Can you work these out from the model? Positions are in its coordinate system, mm. Give positions to 0.01 mm unless a question says otherwise; leave off trailing zeros. Order: outer loops, then holes, each group sorted by start corner. A loop starts at its lowest first (then second) coordinate and runs counter-clockwise, first axis right, second up. Notation, with made-up numbers: (-15, -26) -> (-7, -26) arc R15 ccw to (-7, -5) -> close; hole circle Ø2 at (45, 18). An arc over 180 degrees is marked (long way). Answer as CSV lines item,"result".
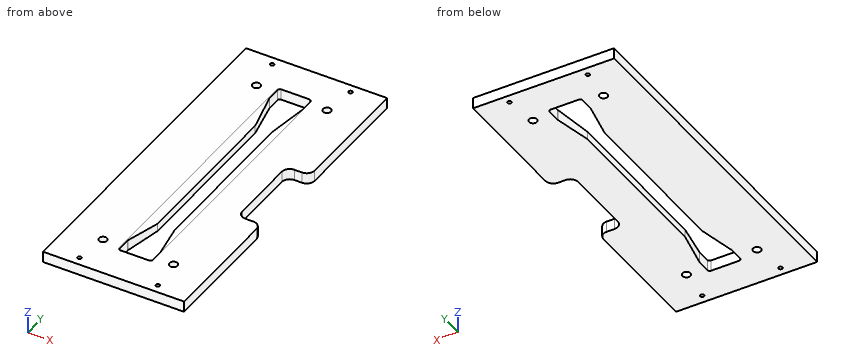
```python
from build123d import *

# Parameters (mm, degrees)
SKETCH1_W              = 180
SKETCH1_H              = 436
BOSS_EXTRUDE1_DEPTH    = 14
SKETCH5_W              = 30
SKETCH5_H              = 105
CUT_EXTRUDE1_DEPTH     = 472.902532309
M12_TAPPED_HOLE1_D     = 10.2
M12_TAPPED_HOLE1_DEPTH = 32.75
M12_TAPPED_HOLE1_TIP   = 3.064389157
FILLET1_R              = 10
M6_TAPPED_HOLE1_D      = 5
M6_TAPPED_HOLE1_DEPTH  = 17
M6_TAPPED_HOLE1_TIP    = 1.502151548
CUT_EXTRUDE2_DEPTH     = 5
CUT_EXTRUDE2_DRAFT     = -70


with BuildPart() as part:
    # Sketch1 → Boss-Extrude1 (new body)
    with BuildSketch(Plane.XY):
        with Locations((90, 218)):
            Rectangle(SKETCH1_W, SKETCH1_H)
        with BuildLine():
            Line((72, 45.5), (108, 45.5))
            ThreePointArc((108, 45.5), (110.121320344, 46.378679656), (111, 48.5))
            Line((111, 48.5), (111, 65.187634121))
            ThreePointArc((111, 65.187634121), (110.98386897, 65.498320406), (110.935649355, 65.805665564))
            Line((110.935649355, 65.805665564), (101, 113))
            Line((101, 113), (101, 323))
            Line((101, 323), (110.935649355, 370.194334436))
            ThreePointArc((110.935649355, 370.194334436), (110.98386897, 370.501679594), (111, 370.812365879))
            Line((111, 370.812365879), (111, 387.5))
            ThreePointArc((111, 387.5), (110.121320344, 389.621320344), (108, 390.5))
            Line((108, 390.5), (72, 390.5))
            ThreePointArc((72, 390.5), (69.878679656, 389.621320344), (69, 387.5))
            Line((69, 387.5), (69, 370.812365879))
            ThreePointArc((69, 370.812365879), (69.01613103, 370.501679594), (69.064350645, 370.194334436))
            Line((69.064350645, 370.194334436), (79, 323))
            Line((79, 323), (79, 113))
            Line((79, 113), (69.064350645, 65.805665564))
            ThreePointArc((69.064350645, 65.805665564), (69.01613103, 65.498320406), (69, 65.187634121))
            Line((69, 65.187634121), (69, 48.5))
            ThreePointArc((69, 48.5), (69.878679656, 46.378679656), (72, 45.5))
        make_face(mode=Mode.SUBTRACT)
    extrude(amount=-BOSS_EXTRUDE1_DEPTH)

    # Sketch5 → Cut-Extrude1 (cut, through all)
    with BuildSketch(Plane.XY):
        with Locations((165, 218)):
            Rectangle(SKETCH5_W, SKETCH5_H)
    extrude(amount=-CUT_EXTRUDE1_DEPTH, mode=Mode.SUBTRACT)

    # M12 Tapped Hole1
    with Locations(Plane(origin=(0, 0, -14), x_dir=(-1, 0, 0), z_dir=(0, 0, -1))):
        with Locations((-135, 383), (-45, 383), (-45, 53), (-135, 53)):
            Hole(M12_TAPPED_HOLE1_D / 2, depth=M12_TAPPED_HOLE1_DEPTH)
            with Locations((0, 0, -(M12_TAPPED_HOLE1_DEPTH + M12_TAPPED_HOLE1_TIP / 2))):  # 118° drill point
                Cone(0, M12_TAPPED_HOLE1_D / 2, M12_TAPPED_HOLE1_TIP, mode=Mode.SUBTRACT)

    # Fillet1
    fillet1_edges = [part.edges().sort_by_distance(p)[0] for p in [
        (150, 165.5, -7),
        (150, 270.5, -7),
        (180, 270.5, -7),
        (180, 165.5, -7),
    ]]
    fillet(fillet1_edges, radius=FILLET1_R)

    # M6 Tapped Hole1
    with Locations(Plane.XY):
        with Locations((40, 425), (140, 425), (40, 11), (140, 11)):
            Hole(M6_TAPPED_HOLE1_D / 2, depth=M6_TAPPED_HOLE1_DEPTH)
            with Locations((0, 0, -(M6_TAPPED_HOLE1_DEPTH + M6_TAPPED_HOLE1_TIP / 2))):  # 118° drill point
                Cone(0, M6_TAPPED_HOLE1_D / 2, M6_TAPPED_HOLE1_TIP, mode=Mode.SUBTRACT)


with BuildPart() as cut_extrude2_tool:
    # Sketch8 → Cut-Extrude2 (with draft: the straight prism first)
    with BuildSketch(Plane.XY):
        with BuildLine():
            ThreePointArc((71, 390.5), (68.878679656, 389.621320344), (68, 387.5))
            Line((68, 387.5), (68, 48.5))
            ThreePointArc((68, 48.5), (68.878679656, 46.378679656), (71, 45.5))
            Line((71, 45.5), (109, 45.5))
            ThreePointArc((109, 45.5), (111.121320344, 46.378679656), (112, 48.5))
            Line((112, 48.5), (112, 387.5))
            ThreePointArc((112, 387.5), (111.121320344, 389.621320344), (109, 390.5))
            Line((109, 390.5), (71, 390.5))
        make_face()
    extrude(amount=-CUT_EXTRUDE2_DEPTH)
    # Cut-Extrude2: the draft: its side faces are tilted about the plane it starts from
    cut_extrude2_sides = [cut_extrude2_tool.faces().sort_by_distance(p)[0] for p in [
        (111.121320344, 389.621320344, -2.5),
        (90, 390.5, -2.5),
        (68.878679656, 389.621320344, -2.5),
        (68, 218, -2.5),
        (68.878679656, 46.378679656, -2.5),
        (90, 45.5, -2.5),
        (111.121320344, 46.378679656, -2.5),
        (112, 218, -2.5),
    ]]
    draft(cut_extrude2_sides, Plane.XY, CUT_EXTRUDE2_DRAFT)


with BuildPart() as part_1:
    add(part.part)

    # Cut-Extrude2: cut by cut_extrude2_tool
    add(cut_extrude2_tool.part, mode=Mode.SUBTRACT)


solid = part_1.part
```
Item 1: Imagine slicing it at C-C, the plane z = -9.5. Give the number of separate pieces and of enclosed holes in the cut face, then the cut area to 3 significant figures.
Numbers:
separate pieces,"1"
enclosed holes,"9"
area,"65,600 mm²"
Item 2: For pin 1 (4 mm diameter, centred on x = 40, y = 425, fed in from -Z), with a flat end and sliding along its axis, tell me the tip position at first contact or that it passes through.
Numbers:
pin 1,"passes through"
Item 3: Imagine slicing it at A-A, the plane y = 383. Please give me the cut outline in (x, z).
Numbers:
outline,"(0, -14) -> (39.9, -14) -> (39.9, 0) -> (0, 0) -> close; (50.1, -14) -> (69, -14) -> (69, -0.36) -> (68, 0) -> (50.1, 0) -> close; (111, -14) -> (129.9, -14) -> (129.9, 0) -> (112, 0) -> (111, -0.36) -> close; (140.1, -14) -> (180, -14) -> (180, 0) -> (140.1, 0) -> close"
Item 4: Please list where these lines run through material, in increasing order: line 1 along X through (y, z) = (425, -10.75); line 2 along Y through (x, z) = (45, -5.25); line 3 along Y through (x, z) = (42, -8.5).
Numbers:
line 1,"x = 0 to 37.5, 42.5 to 137.5, 142.5 to 180"
line 2,"y = 0 to 47.9, 58.1 to 377.9, 388.1 to 436"
line 3,"y = 0 to 9.5, 12.5 to 48.88, 57.12 to 378.88, 387.12 to 423.5, 426.5 to 436"
Item 5: Imagine slicing it at B-B, the plane y = 96. Please give me the cut outline in (x, z).
Numbers:
outline,"(0, -14) -> (75.42, -14) -> (75.42, -2.7) -> (68, 0) -> (0, 0) -> close; (104.58, -14) -> (180, -14) -> (180, 0) -> (112, 0) -> (104.58, -2.7) -> close"
